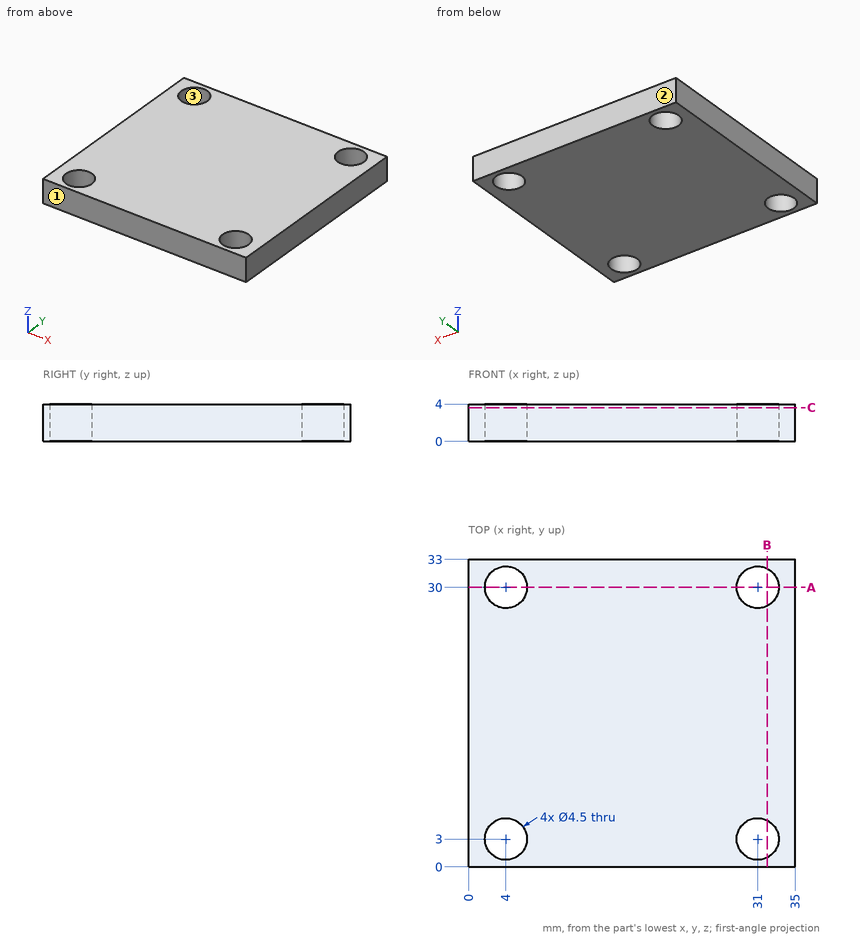
Geometry: see drawing. Coordinates: mm, zero at the bounding-box minimum. Coordinates: 2 decimals unless noted, no trailing zeros. Order: outer loops, then holes, each group sorted by start corner. A loop starts at its lowest first (then second) coordinate and runs counter-clockwise, first axis right, second up. Notation, with made-up numbers: M -17,82 L 37,82 A19 ccw 37,90 Z; hole C -34.75,23.25 d8. An arc over 180 degrees is marked long. Write item = value, one per line. Start each with the question number.
(1) Section C-C on z = 3.6. Output: boundary loops of the cut face in (x, y).
(2) Section B-B on x = 32. Output: boundary loops of the cut face in (y, z).
(3) Pull-direction query (Y, two-part tool) for the marked faces 1, 2 and 3; classes: released by +Y, released by -Y, zero draft, split by the parting line, or undercut.
(4) Line query: line 1 along Y through (x, z) = (4, 2.5); line 2 along Y through (x, z) = (2.5, 1.7); line 3 along X through (y, z) = (28.5, 0.2). Output: solid intervals per line, ascending. Write a range as [from, to].
(5) Section A-A on y = 30. Output: boundary loops of the cut face in (x, z).
Result set:
q1.outline = M 0,0 L 35,0 L 35,33 L 0,33 Z; hole C 4,3 d4.5; hole C 4,30 d4.5; hole C 31,3 d4.5; hole C 31,30 d4.5
q2.outline = M 0,0 L 0.98,0 L 0.98,4 L 0,4 Z; M 5.02,0 L 27.98,0 L 27.98,4 L 5.02,4 Z; M 32.02,0 L 33,0 L 33,4 L 32.02,4 Z
q3.face_1 = released by -Y
q3.face_2 = released by +Y
q3.face_3 = undercut
q4.line_1 = [0, 0.75], [5.25, 27.75], [32.25, 33]
q4.line_2 = [0, 1.32], [4.68, 28.32], [31.68, 33]
q4.line_3 = [0, 2.32], [5.68, 29.32], [32.68, 35]
q5.outline = M 0,0 L 1.75,0 L 1.75,4 L 0,4 Z; M 6.25,0 L 28.75,0 L 28.75,4 L 6.25,4 Z; M 33.25,0 L 35,0 L 35,4 L 33.25,4 Z
